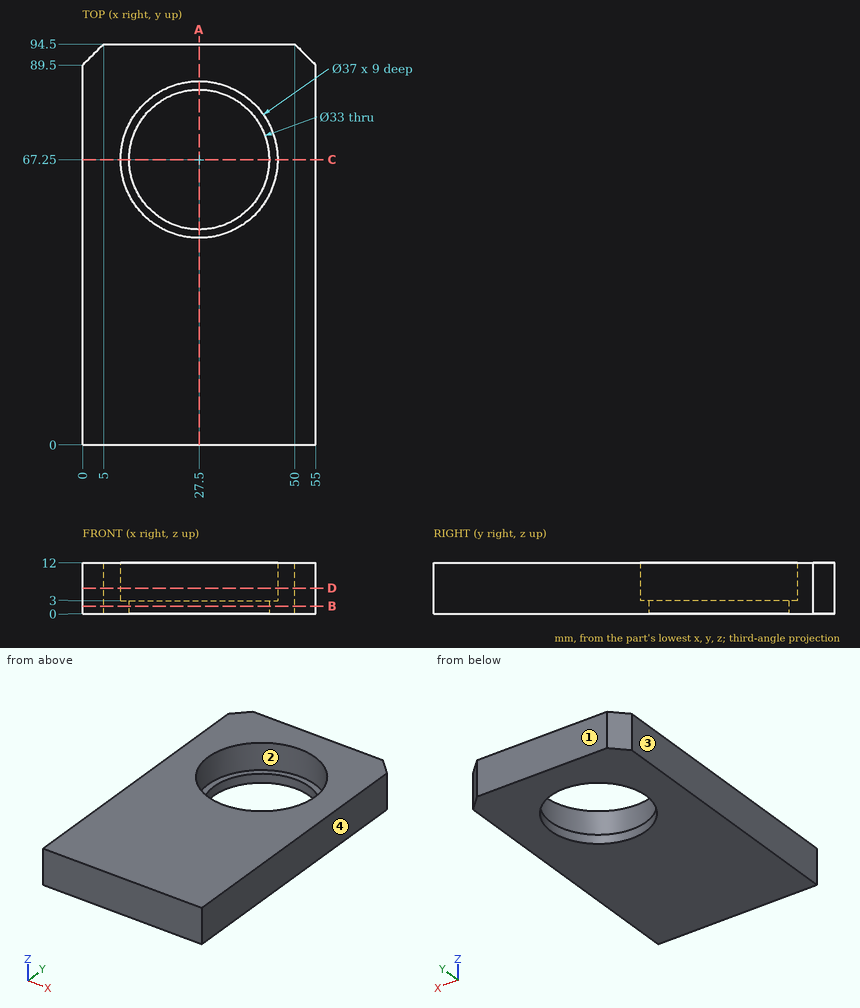
Design review of the part shown in the three views and the two pictorial views. Dimensions are in mm from the part's minimum x, y and z. Give positions to 0.01 mm unless a question says otherwise; leave off trailing zeros. Loops run counter-clockwise (first coordinate to the right, second up) from the corner with the lowest first, then second, coordinate; pieces in that order, holes last. Notation, with made-up numbers: (1.25, -32.75) - (19.25, -32.75) arc R19 ccw to (19.25, 0.25) - close; hole circle Ø9 at (37, 21.25). An arc over 180 degrees is marked (long way). Write item = value, one per line.
1) To check wall thickness, follow line 1 (Y direction, x = 27.5, z = 2); line 2 (Y direction, x = 28, z = 8.75); line 3 (X direction, y = 76.5, z = 7.75). State the ranges of each line that lie inside material, in increasing order.
Result sheet:
line_1 = 0 to 50.75, 83.75 to 94.5
line_2 = 0 to 48.76, 85.74 to 94.5
line_3 = 0 to 11.48, 43.52 to 55
2) Take a section at D-D on z = 6. State the section outline as (x, y) points, and give its area (3 significant figures).
Result sheet:
outline = (0, 0) - (55, 0) - (55, 89.5) - (50, 94.5) - (5, 94.5) - (0, 89.5) - close; hole circle Ø37 at (27.5, 67.25)
area = 4,100 mm2
3) Draft analysis for pull direction X (two halves, no side actions). For the marked faces 1, 2, 3 and 4, state which applies: +X half, -X half, draft (parallel to the pull), parting line (faces both ways), or undercut.
Result sheet:
face_1 = draft
face_2 = undercut
face_3 = -X half
face_4 = +X half
4) Take a section at B-B on z = 1.75. State the section outline as (x, y) points, and give its area (3 significant figures).
Result sheet:
outline = (0, 0) - (55, 0) - (55, 89.5) - (50, 94.5) - (5, 94.5) - (0, 89.5) - close; hole circle Ø33 at (27.5, 67.25)
area = 4,320 mm2
5) Take a section at C-C on y = 67.25. State the section outline as (x, z) points.
Result sheet:
outline = (0, 0) - (11, 0) - (11, 3) - (9, 3) - (9, 12) - (0, 12) - close; (44, 0) - (55, 0) - (55, 12) - (46, 12) - (46, 3) - (44, 3) - close
6) Take a section at A-A on x = 27.5. State the section outline as (y, z) points, and give its area (3 significant figures).
Result sheet:
outline = (0, 0) - (50.75, 0) - (50.75, 3) - (48.75, 3) - (48.75, 12) - (0, 12) - close; (83.75, 0) - (94.5, 0) - (94.5, 12) - (85.75, 12) - (85.75, 3) - (83.75, 3) - close
area = 702 mm2
